```python
from build123d import *

# Parameters (mm, degrees)
EXTRUDE_1_DEPTH = 10


with BuildPart() as part:
    # 草图2 → 拉伸-薄壁1 (new body)
    with BuildSketch(Plane.XY):
        with BuildLine():
            Line((245.832281676, 176.176927505), (27.081748613, -28.88898874))
            ThreePointArc((27.081748613, -28.88898874), (-15.038455107, -36.631129472), (-39.568477007, -1.526566661))
            Line((-39.568477007, -1.526566661), (-47.587213234, 206.31838899))
            ThreePointArc((-47.587213234, 206.31838899), (-0.748703771, 251.498299345), (38.852898358, 199.857391364))
            Line((38.852898358, 199.857391364), (22.971322702, 116.275878645))
            ThreePointArc((22.971322702, 116.275878645), (57.994709331, 76.439587045), (88.052734333, 120.144081921))
            Line((88.052734333, 120.144081921), (64.413334144, 194.838609646))
            ThreePointArc((64.413334144, 194.838609646), (70.809318853, 233.773803242), (106, 251.619639764))
            Line((106, 251.619639764), (216, 251.619639764))
            ThreePointArc((216, 251.619639764), (256.563431385, 224.039981525), (245.832281676, 176.176927505))
        make_face()
        with BuildLine():
            Line((242.412688823, 179.824719264), (23.66215576, -25.241196981))
            ThreePointArc((23.66215576, -25.241196981), (-13.139560233, -32.00574319), (-34.572193971, -1.333808191))
            Line((-34.572193971, -1.333808191), (-42.590930198, 206.511147461))
            ThreePointArc((-42.590930198, 206.511147461), (-1.121390965, 246.512208266), (33.940787828, 200.790756321))
            Line((33.940787828, 200.790756321), (18.059212172, 117.209243602))
            ThreePointArc((18.059212172, 117.209243602), (58.291367675, 71.448395421), (92.819700095, 121.652736099))
            Line((92.819700095, 121.652736099), (69.180299905, 196.347263824))
            ThreePointArc((69.180299905, 196.347263824), (74.843130382, 230.819422671), (106, 246.619639764))
            Line((106, 246.619639764), (216, 246.619639764))
            ThreePointArc((216, 246.619639764), (251.913756192, 222.201362315), (242.412688823, 179.824719264))
        make_face(mode=Mode.SUBTRACT)
    extrude(amount=EXTRUDE_1_DEPTH)


solid = part.part
```
Verification items for the finished model (mm, model axes). A direction names the side the tool comes from. Round coordinates to 2 decimals unless told otherwise and drop trailing zeros. Write each loop counter-clockwise with the first axis right and the second up, starting at its lowest first coordinate (ties: lowest second). Pieces come first, ordered by that corner, then holes. Notation, with made-up numbers: (84, 55) -> (95, 55) arc R16 ccw to (95, 59) -> close; hole circle Ø9 at (-5, -24). An arc over 180 degrees is marked (long way). Write each question's results on one line, items separated by ' | '.
Q1. Access from +Z, -Z, +X, -X, +Y, -Y to the whole of each face (thin tool, end or side, straight path). Record for faces 1 (the face through (74.546, 230.408, 4.93)), 2 (the face through (84, 139, 0)).
Derived:
face 1: +Z, -Z | face 2: -Z, +X, -X, +Y, -Y
Q2. Sectioned sample at B-B, the plane x = 238.5. Record the boundary of the cut face in (y, z), and give its area (3 significant figures).
Derived:
outline: (169.3, 0) -> (176.16, 0) -> (176.16, 10) -> (169.3, 10) -> close; (239.39, 0) -> (245.37, 0) -> (245.37, 10) -> (239.39, 10) -> close | area: 128 mm²
Q3. Sectioned sample at A-A, the plane z = 3.75. Record the boundary of the cut face in (x, y).
Derived:
outline: (-47.59, 206.32) -> (-39.57, -1.53) arc R39.6 ccw to (27.08, -28.89) -> (245.83, 176.18) arc R43.62 ccw to (216, 251.62) -> (106, 251.62) arc R43.62 ccw to (64.41, 194.84) -> (88.05, 120.14) arc R33.62 cw (long way) to (22.97, 116.28) -> (38.85, 199.86) arc R43.62 ccw (long way) to start; hole (-42.59, 206.51) -> (-34.57, -1.33) arc R34.6 ccw to (23.66, -25.24) -> (242.41, 179.82) arc R38.62 ccw to (216, 246.62) -> (106, 246.62) arc R38.62 ccw to (69.18, 196.35) -> (92.82, 121.65) arc R38.62 cw (long way) to (18.06, 117.21) -> (33.94, 200.79) arc R38.62 ccw (long way) to start
Q4. Sectioned sample at C-C, the plane y = 110. Record the boundary of the cut face in (x, z), and give its area (3 significant figures).
Derived:
outline: (-43.87, 0) -> (-38.87, 0) -> (-38.87, 10) -> (-43.87, 10) -> close; (17.38, 0) -> (22.38, 0) -> (22.38, 10) -> (17.38, 10) -> close; (89.62, 0) -> (94.62, 0) -> (94.62, 10) -> (89.62, 10) -> close; (167.93, 0) -> (175.24, 0) -> (175.24, 10) -> (167.93, 10) -> close | area: 223 mm²
Q5. Sectioned sample at D-D, the plane x = 2.5. Record the boundary of the cut face in (y, z), and give its area (3 significant figures).
Derived:
outline: (-39.52, 0) -> (-34.51, 0) -> (-34.51, 10) -> (-39.52, 10) -> close; (246.07, 0) -> (251.13, 0) -> (251.13, 10) -> (246.07, 10) -> close | area: 101 mm²
Q6. Draft check along X on faces 3 (the face through (84, 139, 10)), 4 (the face through (-12.63, -32.21, 4.93)), 5 (the face through (-14.451, -36.867, 4.93)). Enter one of: released by +X, released by -X, zero draft, split by the parting line, or undercut.
Derived:
face 3: zero draft | face 4: undercut | face 5: split by the parting line
Q7. Go/stop test with flat-tipped pins: pin 1 Ø3 at (y, z) = (160.5, 6.5) entering from +X; pin 2 Ø3 at (x, z) = (188, 3.5) entering from -Y; pin 3 Ø2 at (y, z) = (91.5, 3) entering from +X. Record where each tip stops, or that it passes through.
Derived:
pin 1: stops at x = 230.71 | pin 2: stops at y = 120.56 | pin 3: stops at x = 156.57
Q8. Thickness scan on probe 1 along X at (y, z) = (110, 4); probe 2 along X at (y, z) = (208, 4); probe 3 along Y at (x, z) = (95, 3.5). Record the ranges inside material, lowest first.
Derived:
probe 1: x = -43.87 to -38.87, 17.38 to 22.38, 89.62 to 94.62, 167.93 to 175.24 | probe 2: x = -47.62 to -42.62, 34.62 to 39.62, 62.38 to 67.38, 254.62 to 259.62 | probe 3: y = 34.78 to 41.63, 245.02 to 250.21
